Answer from the drawing. Dimensions are ordinates in mm from the lowest x, y and z of the part. A direction names the side the tool comes from. Give positions to 0.01 mm unless a question says otherwise; leave off trailing zeros. Write each loop counter-clockwise with the first axis right and the second up, starting at its lowest first coordinate (ties: lowest second). Pieces come first, ordered by that corner, then holes. Notation, with made-up numbers: (63, 89) - (89, 89) arc R20 cw to (89, 125) - close; hole circle Ø9 at (-1, -25). An arc over 180 degrees is marked (long way). Answer as a JSON object with one key per item and string values. Group by question number.
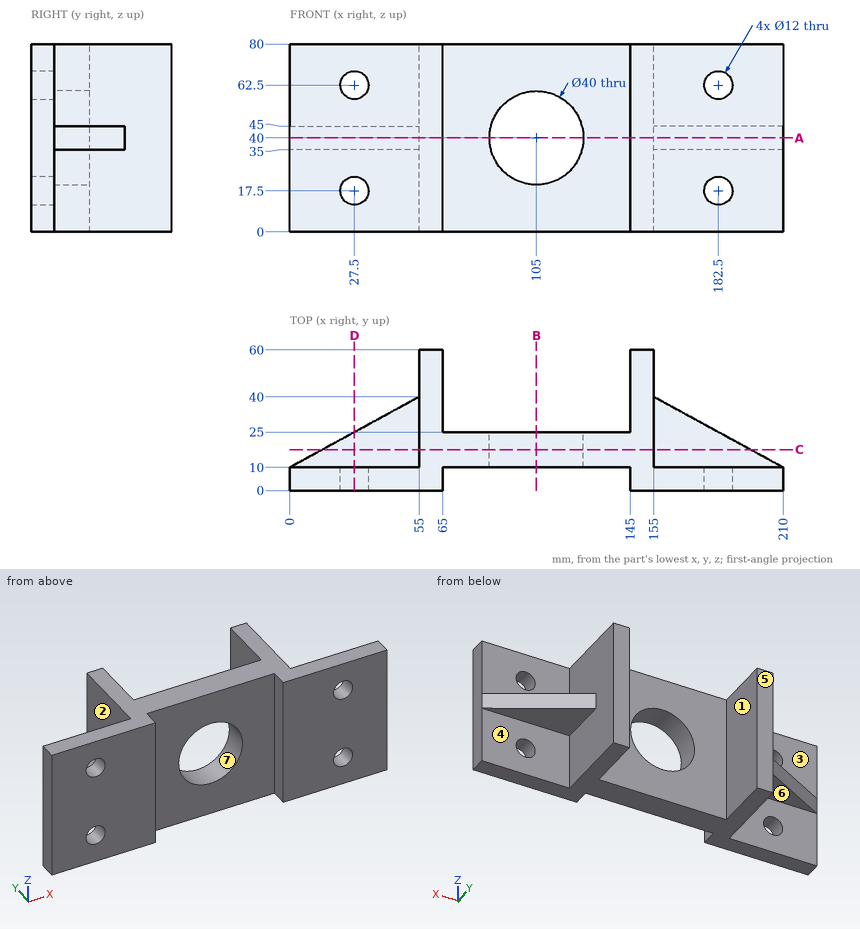
1) For a pull along Z with two mould halves and no side action, classify the marked faces 5, 6 and 7 as released by +Z, released by -Z, zero draft, split by the parting line, or undercut.
2) Find the intervals of material crossed by line 1 (X direction, y = 2.75, z = 62.5); line 2 (X direction, y = 4, z = 19); line 3 (X direction, y = 52, z = 4), in increasing order. Write a range as [from, to].
3) Find section B-B, the plane x = 105. Write down the section's boundary in (y, z), and give its area (3 significant figures).
4) Find section D-D, the plane x = 27.5. Write down the section's boundary in (y, z), and give its area (3 significant figures).
5) Which of the six approach directions +Z, -Z, +X, -X, +Y, -Y give full straight-line access (tool end or side, diameter ignored) to the marked faces 1, 2, 3 and 4?
6) Find section A-A, the plane z = 40. Write down the section's boundary in (x, y).
7) Find section C-C, the plane y = 17.5. Write down the section's boundary in (x, z).
8) Flat-ended cylindrical pins translate along their axes: pin 1 Ø3 at (x, y) = (136, 23) entering from -Z; pin 2 Ø1.5 at (y, z) = (41.5, 21) entering from +X; pin 3 Ø2 at (x, y) = (36, 12) entering from -Z; pin 4 Ø12 at (x, z) = (123.5, 28.5) entering from -Y. Find the tip coordinate at first contact, or state that the pin passes through.
Values follow:
{
 "1": {"face 5": "zero draft", "face 6": "released by -Z", "face 7": "undercut"},
 "2": {"line 1": "x = [0, 21.5], [33.5, 65], [145, 176.5], [188.5, 210]", "line 2": "x = [0, 21.69], [33.31, 65], [145, 176.69], [188.31, 210]", "line 3": "x = [55, 65], [145, 155]"},
 "3": {"outline": "(10, 0) - (25, 0) - (25, 20) - (10, 20) - close; (10, 60) - (25, 60) - (25, 80) - (10, 80) - close", "area": "600 mm2"},
 "4": {"outline": "(0, 0) - (10, 0) - (10, 11.5) - (0, 11.5) - close; (0, 23.5) - (10, 23.5) - (10, 35) - (25, 35) - (25, 45) - (10, 45) - (10, 56.5) - (0, 56.5) - close; (0, 68.5) - (10, 68.5) - (10, 80) - (0, 80) - close", "area": "710 mm2"},
 "5": {"face 1": "+Z, -Z, +Y", "face 2": "-X, +Y", "face 3": "+Z, -X, +Y", "face 4": "-Z, +X, +Y"},
 "6": {"outline": "(0, 0) - (65, 0) - (65, 10) - (85, 10) - (85, 25) - (65, 25) - (65, 60) - (55, 60) - (55, 40) - (0, 10) - close; (125, 10) - (145, 10) - (145, 0) - (210, 0) - (210, 10) - (155, 40) - (155, 60) - (145, 60) - (145, 25) - (125, 25) - close"},
 "7": {"outline": "(13.75, 35) - (55, 35) - (55, 0) - (155, 0) - (155, 35) - (196.25, 35) - (196.25, 45) - (155, 45) - (155, 80) - (55, 80) - (55, 45) - (13.75, 45) - close; hole circle Ø40 at (105, 40)"},
 "8": {"pin 1": "stops at z = 0", "pin 2": "stops at x = 155", "pin 3": "stops at z = 35", "pin 4": "stops at y = 10"}
}
